Check sheet for the modelled part. Datum: model origin and axes. Units: mm. Give positions to 0.01 mm unless a question says otherwise; leave off trailing zeros. Loops run counter-clockwise (first coordinate to the right, second up) from the corner with the lowest first, then second, coordinate; pieces in that order, holes last. Notation, with made-up numbers: M 70,43.5 L 84,43.5 A14 ccw 84,51.5 Z; hole C 32,89.25 d7. An arc over 180 degrees is marked long. One line per question, with ' | ' between items. Start each with the question number.
from build123d import *

# Parameters (mm, degrees)
SKETCH_1_W              = 100
SKETCH_1_H              = 50
EXTRUDE_1_DEPTH         = 12
HOLE_WIZARD_8_5_8_5_1_D = 8.5
CHAMFER_1_SIZE          = 5


with BuildPart() as part:
    # 草图1 → 凸台-拉伸1 (new body)
    with BuildSketch(Plane(origin=(0, 0, 0), x_dir=(0, 0, -1), z_dir=(1, 0, 0))):
        Rectangle(SKETCH_1_W, SKETCH_1_H)
    extrude(amount=EXTRUDE_1_DEPTH)

    # Ø8.5 (8.5) 直径孔1 (through all)
    with Locations(Plane(origin=(12, 0, 0), x_dir=(0, 0, -1), z_dir=(1, 0, 0))):
        with Locations((-40, 15), (-40, -15), (40, 15), (40, -15)):
            Hole(HOLE_WIZARD_8_5_8_5_1_D / 2)

    # 倒角1
    chamfer_1_edges = [part.edges().sort_by_distance(p)[0] for p in [
        (6, -25, -50),
        (6, -25, 50),
        (6, 25, 50),
        (6, 25, -50),
    ]]
    chamfer(chamfer_1_edges, length=CHAMFER_1_SIZE)


solid = part.part
Q1. Cross-section at B-B (x = 2.75). Record the cut outline in (y, z), and give its area (3 significant figures).
Q2. Cross-section at A-A (z = -40). Record the cut outline in (x, y).
Q3. Depth check by flat-ended pin: P1, Ø7.5, axis at y = -15, z = 40, coming from the -X side. Enter the tip coordinate at first touch or a pass-through.
Q4. Material ranges on probe 1 along Z at (x, y) = (6.25, -16.5); probe 2 along Y at (x, z) = (10, 39); probe 3 along Z at (x, y) = (1.25, 12.5), recorded low to high. Write a range as from..to.
Q5. Cross-section at C-C (y = 15). Record the cut outline in (x, z), and give its area (3 significant figures).
Q6. Draft check along Z on faces 1 (the cylindrical face through (5.916, -14.813, -44.246)), 2 (the flat face through (6, 0, -50)), 3 (the cylindrical face through (5.916, 15.187, 35.754)), 4 (the flat face through (6, 23, 47)). Enter one of: released by +Z, released by -Z, zero draft, split by the parting line, or undercut.
Solved:
1) outline: M -25,-45 L -20,-50 L 20,-50 L 25,-45 L 25,45 L 20,50 L -20,50 L -25,45 Z; hole C -15,-40 d8.5; hole C -15,40 d8.5; hole C 15,-40 d8.5; hole C 15,40 d8.5 | area: 4,720 mm²
2) outline: M 0,-25 L 12,-25 L 12,-19.25 L 0,-19.25 Z; M 0,-10.75 L 12,-10.75 L 12,10.75 L 0,10.75 Z; M 0,19.25 L 12,19.25 L 12,25 L 0,25 Z
3) P1: passes through
4) probe 1: z = -50..-43.98, -36.02..36.02, 43.98..50 | probe 2: y = -25..-19.13, -10.87..10.87, 19.13..25 | probe 3: z = -50..-43.44, -36.56..36.56, 43.44..50
5) outline: M 0,-50 L 12,-50 L 12,-44.25 L 0,-44.25 Z; M 0,-35.75 L 12,-35.75 L 12,35.75 L 0,35.75 Z; M 0,44.25 L 12,44.25 L 12,50 L 0,50 Z | area: 996 mm²
6) face 1: undercut | face 2: released by -Z | face 3: undercut | face 4: released by +Z
